Work out the finished part from the listing and answer in its coordinate system (mm). Face numbers are marked on the shaded views. A direction names the side the tool comes from. Round coordinates to 2 decimals unless told otherwise and drop trailing zeros. Loops run counter-clockwise (first coordinate to the right, second up) from the corner with the lowest first, then second, coordinate; pieces in that order, holes last. Notation, with made-up numbers: (14, 68.25) -> (20, 68.25) arc R21 ccw to (20, 83.25) -> close; hole circle Ø6 at (-33, 24.5). An arc over 180 degrees is marked (long way). Write item = value, one per line. Start each with the question number.
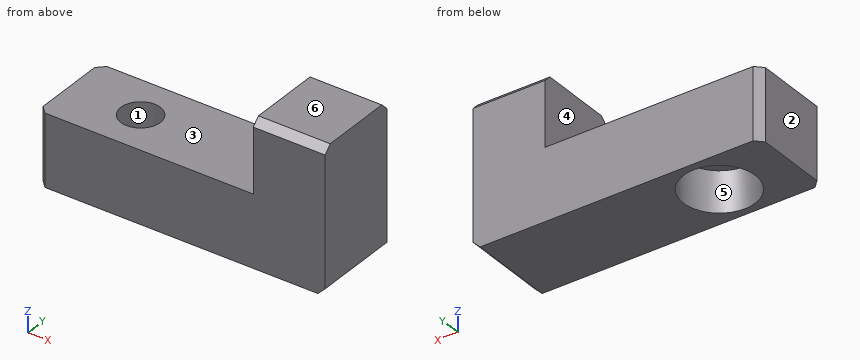
```python
from build123d import *

# Parameters (mm, degrees)
SKETCH_1_W                = 40
SKETCH_1_H                = 20
EXTRUDE_1_DEPTH           = 6
SKETCH_2_W                = 30
SKETCH_2_H                = 10
CUT_EXTRUDE_1_DEPTH       = 12
HOLE_WIZARD_1_D           = 5.5
HOLE_WIZARD_1_CBORE_D     = 10
HOLE_WIZARD_1_CBORE_DEPTH = 5.7
CHAMFER_1_SIZE            = 1


with BuildPart() as part:
    # 草图1 → 凸台-拉伸1 (new, symmetric)
    with BuildSketch(Plane(origin=(0, 0, 0), x_dir=(1, 0, 0), z_dir=(0, 1, 0))):
        Rectangle(SKETCH_1_W, SKETCH_1_H)
    extrude(amount=EXTRUDE_1_DEPTH, both=True)

    # 草图2 → 切除-拉伸1 (cut)
    with BuildSketch(Plane(origin=(0, 6, 0), x_dir=(1, 0, 0), z_dir=(0, 1, 0))):
        with Locations((-5, -5)):
            Rectangle(SKETCH_2_W, SKETCH_2_H)
    extrude(amount=-CUT_EXTRUDE_1_DEPTH, mode=Mode.SUBTRACT)

    # 打孔尺寸(%根据)内六角圆柱头螺钉的类型1 (through all)
    with Locations(Plane(origin=(0, 0, -10), x_dir=(-1, 0, 0), z_dir=(0, 0, -1))):
        with Locations((10, 0)):
            CounterBoreHole(HOLE_WIZARD_1_D / 2, HOLE_WIZARD_1_CBORE_D / 2, HOLE_WIZARD_1_CBORE_DEPTH)

    # 倒角1
    chamfer_1_edges = [part.edges().sort_by_distance(p)[0] for p in [
        (-20, 6, -5),
        (15, -6, 10),
        (15, 6, 10),
        (-20, -6, -5),
        (20, 0, -10),
    ]]
    chamfer(chamfer_1_edges, length=CHAMFER_1_SIZE)


solid = part.part
```
Item 1: Section C-C (x = -10) is taken. Determine the outline of the cut face in (y, z), then the cut area to 4 significant figures.
Item 2: Section D-D (z = -2) is taken. Determine the outline of the cut face in (x, y).
Item 3: Section B-B (z = -5.25) is taken. Determine the outline of the cut face in (x, y).
Item 4: Find the intervals of material crossed by line 1 along Y through (x, z) = (-10, -2.55); line 2 along Y through (x, z) = (-10, -6.9); line 3 along Z through (x, y) = (6.5, 2.5), in increasing order. Write a range as [from, to].
Item 5: Section A-A (y = 0) is taken. Determine the outline of the cut face in (x, z).
Item 6: Flat-ended cylindrical pins translate along their axes: pin 1 (3 mm diameter, centred on y = -1.5, z = 7.5, fed in from -X); pin 2 (6.5 mm diameter, centred on x = -10, y = 0, fed in from +Z); pin 3 (6 mm diameter, centred on x = -10, y = 0, fed in from -Z). Find the tip coordinate at first contact, or state that the pin passes through.
Item 7: The mould has two halves that part along X. Classify the marked faces 1, 2 and 3: pulls with the +X half, pulls with the -X half, needs draft (parallel to the pull), parting line crosses it, or undercut.
Item 8: A tool of negligible diameter and unlimited length cuts with its end or side. For the marked faces 4, 5 and 6, from which of +Z, -Z, +X, -X, +Y, -Y can it reach the whole face along a straight path? Write none if from no direction.
Worked answers:
q1.outline = (-6, -10) -> (-5, -10) -> (-5, -4.3) -> (-2.75, -4.3) -> (-2.75, 0) -> (-6, 0) -> close; (2.75, -4.3) -> (5, -4.3) -> (5, -10) -> (6, -10) -> (6, 0) -> (2.75, 0) -> close
q1.area = 39.35 mm2
q2.outline = (-20, -5) -> (-19, -6) -> (20, -6) -> (20, 6) -> (-19, 6) -> (-20, 5) -> close; hole circle Ø5.5 at (-10, 0)
q3.outline = (-20, -5) -> (-19, -6) -> (20, -6) -> (20, 6) -> (-19, 6) -> (-20, 5) -> close; hole circle Ø10 at (-10, 0)
q4.line_1 = [-6, -2.75], [2.75, 6]
q4.line_2 = [-6, -5], [5, 6]
q4.line_3 = [-10, 0]
q5.outline = (-20, -10) -> (-15, -10) -> (-15, -4.3) -> (-12.75, -4.3) -> (-12.75, 0) -> (-20, 0) -> close; (-7.25, -4.3) -> (-5, -4.3) -> (-5, -10) -> (19, -10) -> (20, -9) -> (20, 10) -> (10, 10) -> (10, 0) -> (-7.25, 0) -> close
q6.pin_1 = 10
q6.pin_2 = 0
q6.pin_3 = -4.3
q7.face_1 = undercut
q7.face_2 = pulls with the -X half
q7.face_3 = needs draft
q8.face_4 = +Z, -X, +Y, -Y
q8.face_5 = -Z
q8.face_6 = +Z, +X, -X, +Y, -Y
